Geometry check sheet. Reference: the model listing, model coordinates, mm. Face numbers are marked on the shaded views. A direction names the side the tool comes from. Round coordinates to 2 decimals unless told otherwise and drop trailing zeros. Write each loop counter-clockwise with the first axis right and the second up, starting at its lowest first coordinate (ties: lowest second). Pieces come first, ordered by that corner, then holes. Notation, with made-up numbers: (-26.5, 75) - (-7.5, 75) arc R12 ccw to (-7.5, 88) - close; hole circle Ø10 at (6.5, 24.25). An arc over 180 degrees is marked (long way). Return JSON: item names as keys, results as strings. Group by question number.
from build123d import *

# Parameters (mm, degrees)
SKETCH1_W                                            = 15
SKETCH1_H                                            = 10
BOSS_EXTRUDE1_DEPTH                                  = 7
SKETCH2_W                                            = 9
SKETCH2_H                                            = 15.767491366
CUT_EXTRUDE1_DEPTH                                   = 3
SKETCH4_W                                            = 6
SKETCH4_H                                            = 5
CUT_EXTRUDE3_DEPTH                                   = 6
HOLE_SIZE_PER_SOCKET_HEAD_CAP_SCREW_TYPE_D           = 3.4
HOLE_SIZE_PER_SOCKET_HEAD_CAP_SCREW_TYPE_CBORE_D     = 6
HOLE_SIZE_PER_SOCKET_HEAD_CAP_SCREW_TYPE_CBORE_DEPTH = 3.4
FILLET1_R                                            = 2


with BuildPart() as part:
    # Sketch1 → Boss-Extrude1 (new body)
    with BuildSketch(Plane.XY):
        Rectangle(SKETCH1_W, SKETCH1_H)
    extrude(amount=BOSS_EXTRUDE1_DEPTH)

    # Sketch2 → Cut-Extrude1 (cut)
    with BuildSketch(Plane.XY.offset(7)):
        Rectangle(SKETCH2_W, SKETCH2_H)
    extrude(amount=-CUT_EXTRUDE1_DEPTH, mode=Mode.SUBTRACT)

    # Sketch4 → Cut-Extrude3 (cut)
    with BuildSketch(Plane(origin=(0, 0, 0), x_dir=(-1, 0, 0), z_dir=(0, 0, -1))):
        with Locations((-7.5, 0)):
            Rectangle(SKETCH4_W, SKETCH4_H)
        with Locations((7.5, 0)):
            Rectangle(SKETCH4_W, SKETCH4_H)
    extrude(amount=-CUT_EXTRUDE3_DEPTH, mode=Mode.SUBTRACT)

    # Hole size per socket head cap screw type 1 (through all)
    with Locations(Plane.XY.offset(4)):
        with Locations((0, 0)):
            CounterBoreHole(HOLE_SIZE_PER_SOCKET_HEAD_CAP_SCREW_TYPE_D / 2, HOLE_SIZE_PER_SOCKET_HEAD_CAP_SCREW_TYPE_CBORE_D / 2, HOLE_SIZE_PER_SOCKET_HEAD_CAP_SCREW_TYPE_CBORE_DEPTH)

    # Fillet1
    fillet1_edges = [part.edges().sort_by_distance(p)[0] for p in [
        (7.5, -5, 3.5),
        (-7.5, -5, 3.5),
        (-7.5, 5, 3.5),
        (7.5, 5, 3.5),
    ]]
    fillet(fillet1_edges, radius=FILLET1_R)


solid = part.part
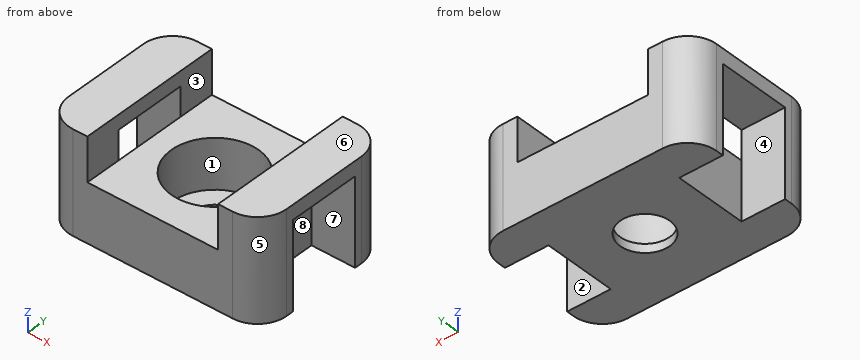
1. Mould release check, pull along Y, two halves, no side actions. Record for the marked faces 5, 6, 7 and 8: pulls with the +Y half, pulls with the -Y half, needs draft (parallel to the pull), parting line crosses it, or undercut.
2. Section check A-A (z = 6.75). Enter the section's corners in (x, y), and give its area (3 significant figures).
3. Tool access check on the marked faces 1, 2, 3 and 4. Record the directions out of +Z, -Z, +X, -X, +Y, -Y that give a thin tool (end or side, any length) a straight path to the whole face; none if there is none.
4. Material ranges on line 1 along Y through (x, z) = (0, 2.7); line 2 along X through (y, z) = (2.75, 6); line 3 along Y through (x, z) = (0, 0.4), recorded low to high.
5. Section check D-D (y = 0). Enter the section's corners in (x, z), and give its area (3 significant figures).
6. Section check B-B (z = 4.5). Enter the section's corners in (x, y), and give its area (3 significant figures).
7. Section check C-C (x = 0). Enter the section's corners in (y, z), and give its area (3 significant figures).
8. Depth check by flat-ended pin: pin 1 Ø0.9 at (y, z) = (0.5, 5) entering from +X; pin 2 Ø1.5 at (x, z) = (-6.5, 3) entering from +Y; pin 3 Ø5 at (x, y) = (1, -0.5) entering from +Z; pin 4 Ø2.5 at (x, y) = (6, 1) entering from -Z. Enter the tip coordinate at first touch or a pass-through.
Result sheet:
{
 "1": {"face 5": "pulls with the -Y half", "face 6": "needs draft", "face 7": "undercut", "face 8": "undercut"},
 "2": {"outline": "(-7.5, -3) arc R2 ccw to (-5.5, -5) - (-4.5, -5) - (-4.5, 5) - (-5.5, 5) arc R2 ccw to (-7.5, 3) - close; (4.5, -5) - (5.5, -5) arc R2 ccw to (7.5, -3) - (7.5, 3) arc R2 ccw to (5.5, 5) - (4.5, 5) - close", "area": "56.6 mm²"},
 "3": {"face 1": "+Z", "face 2": "-Z, +X", "face 3": "+Z, +Y, -Y", "face 4": "-Z, -X"},
 "4": {"line 1": "y = -5 to -3, 3 to 5", "line 2": "x = -7.5 to -4.5, 4.5 to 7.5", "line 3": "y = -5 to -1.7, 1.7 to 5"},
 "5": {"outline": "(-7.5, 6) - (-4.5, 6) - (-4.5, 7) - (-7.5, 7) - close; (-4.5, 0) - (-1.7, 0) - (-1.7, 0.6) - (-3, 0.6) - (-3, 4) - (-4.5, 4) - close; (1.7, 0) - (4.5, 0) - (4.5, 4) - (3, 4) - (3, 0.6) - (1.7, 0.6) - close; (4.5, 6) - (7.5, 6) - (7.5, 7) - (4.5, 7) - close", "area": "19.6 mm²"},
 "6": {"outline": "(-7.5, -3) arc R2 ccw to (-5.5, -5) - (-4.5, -5) - (-4.5, -2.5) - (-7.5, -2.5) - close; (-7.5, 2.5) - (-4.5, 2.5) - (-4.5, 5) - (-5.5, 5) arc R2 ccw to (-7.5, 3) - close; (4.5, -5) - (5.5, -5) arc R2 ccw to (7.5, -3) - (7.5, -2.5) - (4.5, -2.5) - close; (4.5, 2.5) - (7.5, 2.5) - (7.5, 3) arc R2 ccw to (5.5, 5) - (4.5, 5) - close", "area": "26.6 mm²"},
 "7": {"outline": "(-5, 0) - (-1.7, 0) - (-1.7, 0.6) - (-3, 0.6) - (-3, 4) - (-5, 4) - close; (1.7, 0) - (5, 0) - (5, 4) - (3, 4) - (3, 0.6) - (1.7, 0.6) - close", "area": "17.6 mm²"},
 "8": {"pin 1": "passes through", "pin 2": "stops at y = 4.98", "pin 3": "stops at z = 4", "pin 4": "stops at z = 6"}
}
